Source: CAD feature listing. Evaluate the final solid. Frame: model axes, mm. Face numbers are marked on the shaded views. Round coordinates to 2 decimals unless told otherwise and drop trailing zeros. Write each loop counter-clockwise with the first axis right and the second up, starting at its lowest first coordinate (ties: lowest second). Pieces come first, ordered by that corner, then holes. Notation, with made-up numbers: (63, 9) -> (120, 9) arc R19 cw to (120, 38) -> close; hole circle Ø6 at (26, -7). An arc over 180 degrees is marked (long way). Return JSON: item names as keys, results as strings. Group by question number.
from build123d import *

# Parameters (mm, degrees)
SKETCH1_W             = 97.5
SKETCH1_H             = 45
SKETCH1_R             = 15
SKETCH1_R_2           = 3.4
BOSS_EXTRUDE1_DEPTH   = 10
CUT_EXTRUDE1_REACH    = 109.848
SKETCH2_W             = 20
SKETCH2_H             = 2
M5_TAPPED_HOLE1_D     = 4.2
M5_TAPPED_HOLE1_DEPTH = 12.4
M5_TAPPED_HOLE1_TIP   = 1.2618073
CHAMFER1_SIZE         = 2


with BuildPart() as part:
    # Sketch1 → Boss-Extrude1 (new body)
    with BuildSketch(Plane.XY):
        with Locations((48.75, 22.5)):
            Rectangle(SKETCH1_W, SKETCH1_H)
        with Locations((22.5, 22.5)):
            Circle(SKETCH1_R, mode=Mode.SUBTRACT)
        with Locations((82.5, 37.5)):
            Circle(SKETCH1_R_2, mode=Mode.SUBTRACT)
        with Locations((82.5, 7.5)):
            Circle(SKETCH1_R_2, mode=Mode.SUBTRACT)
    extrude(amount=BOSS_EXTRUDE1_DEPTH)

    # Sketch2 → Cut-Extrude1 (cut, up to next)
    with BuildSketch(Plane(origin=(0, 45, 0), x_dir=(1, 0, 0), z_dir=(0, 1, 0)), mode=Mode.PRIVATE) as cut_extrude1_sk1:
        with Locations((82.5, -9)):
            Rectangle(SKETCH2_W, SKETCH2_H)
    cut_extrude1_tool1 = extrude(cut_extrude1_sk1.sketch, amount=-CUT_EXTRUDE1_REACH, mode=Mode.PRIVATE) & part.part
    add(cut_extrude1_tool1.solids().sort_by_distance((82.5, 45, 9))[0], mode=Mode.SUBTRACT)

    # M5 Tapped Hole1
    with Locations(Plane(origin=(0, 0, 0), x_dir=(-1, 0, 0), z_dir=(0, 0, -1))):
        with Locations((-39.5, 5.5), (-5.5, 5.5), (-5.5, 39.5), (-39.5, 39.5)):
            Hole(M5_TAPPED_HOLE1_D / 2, depth=M5_TAPPED_HOLE1_DEPTH)
            with Locations((0, 0, -(M5_TAPPED_HOLE1_DEPTH + M5_TAPPED_HOLE1_TIP / 2))):  # 118° drill point
                Cone(0, M5_TAPPED_HOLE1_D / 2, M5_TAPPED_HOLE1_TIP, mode=Mode.SUBTRACT)

    # Chamfer1
    chamfer1_edges = [part.edges().sort_by_distance(p)[0] for p in [
        (0, 45, 5),
        (97.5, 45, 5),
        (97.5, 0, 5),
        (0, 0, 5),
    ]]
    chamfer(chamfer1_edges, length=CHAMFER1_SIZE)


solid = part.part
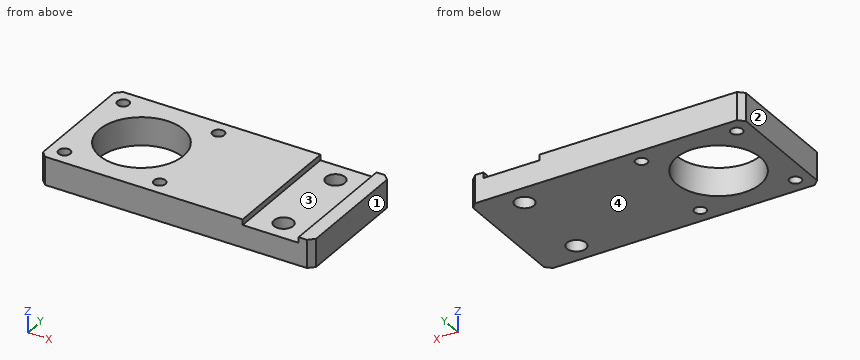
Item 1: Cut plane A-A on x = 82.5. Output: boundary loops of the cut face in (y, z).
Item 2: Cut plane C-C on y = 19. Output: boundary loops of the cut face in (x, z).
Item 3: Cut plane D-D on x = 22.5. Output: boundary loops of the cut face in (y, z).
Item 4: Material intervals for probe 1 along Y at (x, z) = (39.5, 4.25); probe 2 along Y at (x, z) = (82.5, 5); probe 3 along X at (y, z) = (40, 6), sorted ascending.
Item 5: Pull-direction query (X, two-part tool) for the marked faces 1, 2, 3 and 4; classes: +X half, -X half, draft (parallel to the pull), parting line (faces both ways), or undercut.
Item 6: First-contact query: pin 1 Ø2.5 at (x, y) = (39.5, 39.5) entering from +Z; pin 2 Ø11 at (x, y) = (82.5, 37.5) entering from +Z. Flat tips, straight axial feed; report the tip coordinate or a pass-through.
Item 7: Cut plane B-B on z = 3.25. Output: boundary loops of the cut face in (x, y), and give its area (3 significant figures).
Here are the results:
{
 "1": {"outline": "(0, 0) -> (4.1, 0) -> (4.1, 8) -> (0, 8) -> close; (10.9, 0) -> (34.1, 0) -> (34.1, 8) -> (10.9, 8) -> close; (40.9, 0) -> (45, 0) -> (45, 8) -> (40.9, 8) -> close"},
 "2": {"outline": "(0, 0) -> (7.91, 0) -> (7.91, 10) -> (0, 10) -> close; (37.09, 0) -> (97.5, 0) -> (97.5, 10) -> (92.5, 10) -> (92.5, 8) -> (72.5, 8) -> (72.5, 10) -> (37.09, 10) -> close"},
 "3": {"outline": "(0, 0) -> (7.5, 0) -> (7.5, 10) -> (0, 10) -> close; (37.5, 0) -> (45, 0) -> (45, 10) -> (37.5, 10) -> close"},
 "4": {"probe 1": "y = 0 to 3.4, 7.6 to 37.4, 41.6 to 45", "probe 2": "y = 0 to 4.1, 10.9 to 34.1, 40.9 to 45", "probe 3": "x = 0 to 3.46, 7.54 to 37.46, 41.54 to 80.2, 84.8 to 97.5"},
 "5": {"face 1": "+X half", "face 2": "-X half", "face 3": "undercut", "face 4": "draft"},
 "6": {"pin 1": "passes through", "pin 2": "stops at z = 8"},
 "7": {"outline": "(0, 2) -> (2, 0) -> (95.5, 0) -> (97.5, 2) -> (97.5, 43) -> (95.5, 45) -> (2, 45) -> (0, 43) -> close; hole circle Ø4.2 at (5.5, 5.5); hole circle Ø4.2 at (5.5, 39.5); hole circle Ø30 at (22.5, 22.5); hole circle Ø4.2 at (39.5, 5.5); hole circle Ø4.2 at (39.5, 39.5); hole circle Ø6.8 at (82.5, 7.5); hole circle Ø6.8 at (82.5, 37.5)", "area": "3,540 mm^2"}
}
